Verification items for the finished model (mm, model axes). A direction names the side the tool comes from. Give positions to 0.01 mm unless a question says otherwise; leave off trailing zeros. Write each loop counter-clockwise with the first axis right and the second up, starting at its lowest first coordinate (ties: lowest second). Pieces come first, ordered by that corner, then holes.
from build123d import *

# Parameters (mm, degrees)
G1_1_2_TAPPED_HOLE1_D = 45.25
CHAMFER1_SIZE         = 1


with BuildPart() as part:
    # Sketch1 → Revolve1 (revolve)
    with BuildSketch(Plane(origin=(0, 0, 0), x_dir=(0, 0, -1), z_dir=(1, 0, 0)), mode=Mode.PRIVATE) as revolve1_sk:
        Polygon((0, 0), (0, 27.5), (-12, 27.5), (-12, 32.5), (-22, 32.5), (-22, 0), align=None)
    revolve(revolve1_sk.sketch.rotate(Axis((0, 0, 22), (0, 0, -1)), 180), axis=Axis((0, 0, 22), (0, 0, -1)))

    # G1-1/2 Tapped Hole1 (through all)
    with Locations(Plane.XY.offset(22)):
        with Locations((0, 0)):
            Hole(G1_1_2_TAPPED_HOLE1_D / 2)

    # Chamfer1
    chamfer1_edges = [part.edges().sort_by_distance(p)[0] for p in [
        (0, 32.5, 22),
    ]]
    chamfer(chamfer1_edges, length=CHAMFER1_SIZE)


solid = part.part
Item 1: Set-up check for faces 1 (the face through (-9.76, -31, 16.56)), 2 (the face through (24.397, -12.69, 6.084)): record each of +Z, -Z, +X, -X, +Y, -Y from which the full face is reachable in a straight line by a thin tool's end or side.
Answer key:
face 1: +Z, -Z
face 2: -Z
Item 2: Sectioned sample at C-C on z = 13.25. Record the cut outline in (x, y) (3 decimals), then the cut area to 3 significant figures.
Answer key:
outline: circle Ø65 at (0, 0); hole circle Ø45.25 at (0, 0)
area: 1,710 mm2
Item 3: Sectioned sample at A-A on y = 0. Record the cut outline in (x, z) (3 decimals).
Answer key:
outline: (-32.5, 12) - (-27.5, 12) - (-27.5, 0) - (-22.625, 0) - (-22.625, 22) - (-31.5, 22) - (-32.5, 21) - close; (22.625, 0) - (27.5, 0) - (27.5, 12) - (32.5, 12) - (32.5, 21) - (31.5, 22) - (22.625, 22) - close
Item 4: Depth check by flat-ended pin: pin 1 (4 mm diameter, centred on x = 22, y = 14.5, fed in from -Z); pin 2 (12 mm diameter, centred on y = 23.5, z = 3, fed in from +X); pin 3 (2 mm diameter, centred on x = 19.5, z = 14, fed in from -Y); pin 4 (1 mm diameter, centred on y = 9, z = 4.5, fed in from -X). Enter the tip coordinate at first touch or a pass-through.
Answer key:
pin 1: stops at z = 0
pin 2: stops at x = 21.21
pin 3: stops at y = -26.72
pin 4: stops at x = -26.15
Item 5: Scan lines: line 1 along Z through (x, y) = (10, -28.5); line 2 along X through (y, z) = (-5, 11.75); line 3 along X through (y, z) = (20.5, 18.5). Record each from-to range of solid material in increasing order.
Answer key:
line 1: z = 12 to 22
line 2: x = -27.04 to -22.07, 22.07 to 27.04
line 3: x = -25.22 to -9.57, 9.57 to 25.22
